Could you check a few things on this model? Use its own coordinates, in mm. Round coordinates to 2 decimals unless told otherwise and drop trailing zeros. Write each loop counter-clockwise with the first axis right and the second up, starting at its lowest first coordinate (ties: lowest second). Pieces come first, ordered by that corner, then holes. Notation, with made-up numbers: (24, 82.25) -> (44, 82.25) arc R37 cw to (44, 118.25) -> close; hole circle Ø7 at (30, 5). An arc over 180 degrees is marked (long way). Return JSON: item names as keys, results as strings.
from build123d import *

# Parameters (mm, degrees)
SKETCH1_R           = 33.5
SKETCH1_R_2         = 27.5
BOSS_EXTRUDE1_DEPTH = 38.5
CHAMFER1_SIZE       = 1.5


with BuildPart() as part:
    # Sketch1 → Boss-Extrude1 (new body)
    with BuildSketch(Plane(origin=(0, 0, 0), x_dir=(1, 0, 0), z_dir=(0, 1, 0))):
        with Locations(Location((0, 0, 0), (0, 0, 270))):
            Circle(SKETCH1_R)
        with Locations(Location((0, 0, 0), (0, 0, 270))):
            Circle(SKETCH1_R_2, mode=Mode.SUBTRACT)
    extrude(amount=BOSS_EXTRUDE1_DEPTH)

    # Chamfer1
    chamfer1_edges = [part.edges().sort_by_distance(p)[0] for p in [
        (0, 0, -33.5),
        (0, 38.5, -33.5),
        (0, 0, -27.5),
        (0, 38.5, -27.5),
    ]]
    chamfer(chamfer1_edges, length=CHAMFER1_SIZE)


solid = part.part
1) I want a section at A-A, the plane z = 0. Please give me the cut outline in (x, y).
Return value:
{"outline": "(-33.5, 1.5) -> (-32, 0) -> (-29, 0) -> (-27.5, 1.5) -> (-27.5, 37) -> (-29, 38.5) -> (-32, 38.5) -> (-33.5, 37) -> close; (27.5, 1.5) -> (29, 0) -> (32, 0) -> (33.5, 1.5) -> (33.5, 37) -> (32, 38.5) -> (29, 38.5) -> (27.5, 37) -> close"}
2) Will these pins go through, and if not, where does the flat tip stop? pin 1 Ø10 at (y, z) = (14.5, 19.5) entering from +X; pin 2 Ø8 at (x, y) = (-9.5, 6.5) entering from -Z; pin 3 Ø6 at (x, y) = (9.5, 19.5) entering from -Z.
Return value:
{"pin 1": "x = 30.2", "pin 2": "z = -33.05", "pin 3": "z = -32.86"}
3) I want a section at C-C, the plane y = 26.5. Please give me the cut outline in (x, z).
Return value:
{"outline": "circle Ø67 at (0, 0); hole circle Ø55 at (0, 0)"}
4) Thinking about a two-plate mould opening in Z: for faces 1 (the face through (-24.397, 19.002, 12.69)), 2 (the face through (29, 0, -5)), 3 (the face through (-29.7, 19, 15.5)), which applies, pulls with the +Z half, pulls with the -Z half, needs draft (parallel to the pull), parting line crosses it, or undercut?
Return value:
{"face 1": "undercut", "face 2": "needs draft", "face 3": "parting line crosses it"}
5) I want a section at B-B, the plane x = 0. Please give me the cut outline in (y, z).
Return value:
{"outline": "(0, -32) -> (1.5, -33.5) -> (37, -33.5) -> (38.5, -32) -> (38.5, -29) -> (37, -27.5) -> (1.5, -27.5) -> (0, -29) -> close; (0, 29) -> (1.5, 27.5) -> (37, 27.5) -> (38.5, 29) -> (38.5, 32) -> (37, 33.5) -> (1.5, 33.5) -> (0, 32) -> close"}
6) If I drill on probe 1 along X at (y, z) = (29, 0); probe 2 along Z at (x, y) = (-1, 30); probe 3 along Z at (x, y) = (9.5, 34.5), over which ranges is the centre line in solid material (lowest first)? Write a range as [from, to].
Return value:
{"probe 1": "[-33.5, -27.5], [27.5, 33.5]", "probe 2": "[-33.49, -27.48], [27.48, 33.49]", "probe 3": "[-32.12, -25.81], [25.81, 32.12]"}
